Design review of the part built by this model. Coordinates are the model's own, in mm. A direction names the side the tool comes from. Round coordinates to 2 decimals unless told otherwise and drop trailing zeros. Order: outer loops, then holes, each group sorted by start corner. A loop starts at its lowest first (then second) coordinate and runs counter-clockwise, first axis right, second up.
from build123d import *

# Parameters (mm, degrees)
SKETCH1_W           = 32
SKETCH1_H           = 45
BOSS_EXTRUDE1_DEPTH = 8
CUT_EXTRUDE1_DEPTH  = 29.744564704
CUT_EXTRUDE2_DEPTH  = 3.3
FILLET1_R           = 3


with BuildPart() as part:
    # Sketch1 → Boss-Extrude1 (new body)
    with BuildSketch(Plane.XY):
        Rectangle(SKETCH1_W, SKETCH1_H)
    extrude(amount=BOSS_EXTRUDE1_DEPTH)

    # Sketch5 → Cut-Extrude1 (cut, through all)
    with BuildSketch(Plane.XY.offset(8)):
        with BuildLine():
            Line((-8, 1.75), (8, 1.75))
            ThreePointArc((8, 1.75), (9.75, 0), (8, -1.75))
            Line((8, -1.75), (-8, -1.75))
            ThreePointArc((-8, -1.75), (-9.75, 0), (-8, 1.75))
        make_face()
    extrude(amount=-CUT_EXTRUDE1_DEPTH, mode=Mode.SUBTRACT)

    # Sketch6 → Cut-Extrude2 (cut)
    with BuildSketch(Plane.XY.offset(8)):
        with BuildLine():
            Line((-8, 3), (8, 3))
            ThreePointArc((8, 3), (11, 0), (8, -3))
            Line((8, -3), (-8, -3))
            ThreePointArc((-8, -3), (-11, 0), (-8, 3))
        make_face()
    extrude(amount=-CUT_EXTRUDE2_DEPTH, mode=Mode.SUBTRACT)

    # Fillet1
    fillet1_edges = [part.edges().sort_by_distance(p)[0] for p in [
        (-16, 22.5, 4),
        (16, 22.5, 4),
        (16, -22.5, 4),
        (-16, -22.5, 4),
    ]]
    fillet(fillet1_edges, radius=FILLET1_R)


solid = part.part
1) To check wall thickness, follow line 1 along Y through (x, z) = (-3, 6.5); line 2 along Y through (x, z) = (5, 2.5); line 3 along X through (y, z) = (0, 6.5). State the ranges of each line that lie inside material, in increasing order.
Results:
line 1: y = -22.5 to -3, 3 to 22.5
line 2: y = -22.5 to -1.75, 1.75 to 22.5
line 3: x = -16 to -11, 11 to 16
2) Take a section at C-C on x = -5. Give the boundary of the cut face in (y, z).
Results:
outline: (-22.5, 0) - (-1.75, 0) - (-1.75, 4.7) - (-3, 4.7) - (-3, 8) - (-22.5, 8) - close; (1.75, 0) - (22.5, 0) - (22.5, 8) - (3, 8) - (3, 4.7) - (1.75, 4.7) - close
3) Clearance check with a flat-ended pin moving along its axis: P1, Ø3, axis at x = 2.5, y = -0.5, coming from the +Z side. State where the tip first meets the part, or that it passes through.
Results:
P1: stops at z = 4.7
4) Take a section at A-A on z = 7.5. Give the boundary of the cut face in (x, y).
Results:
outline: (-16, -19.5) arc R3 ccw to (-13, -22.5) - (13, -22.5) arc R3 ccw to (16, -19.5) - (16, 19.5) arc R3 ccw to (13, 22.5) - (-13, 22.5) arc R3 ccw to (-16, 19.5) - close; hole (-8, -3) - (8, -3) arc R3 ccw to (8, 3) - (-8, 3) arc R3 ccw to start
5) Take a section at D-D on z = 2.75. Give the boundary of the cut face in (x, y).
Results:
outline: (-16, -19.5) arc R3 ccw to (-13, -22.5) - (13, -22.5) arc R3 ccw to (16, -19.5) - (16, 19.5) arc R3 ccw to (13, 22.5) - (-13, 22.5) arc R3 ccw to (-16, 19.5) - close; hole (-8, -1.75) - (8, -1.75) arc R1.75 ccw to (8, 1.75) - (-8, 1.75) arc R1.75 ccw to start
6) The part is to be moulded in two halves that separate along Y. For faces 4 (the face through (16, 0, 4)), 5 (the face through (15.1, 21.64, 4.06)), 6 (the face through (0, -22.5, 4)), 7 (the face through (0, 3, 6)), say which applies: released by +Y, released by -Y, zero draft, split by the parting line, or undercut.
Results:
face 4: zero draft
face 5: released by +Y
face 6: released by -Y
face 7: undercut
7) Take a section at B-B on y = 0. Give the boundary of the cut face in (x, z), plus the area to 4 significant figures.
Results:
outline: (-16, 0) - (-9.75, 0) - (-9.75, 4.7) - (-11, 4.7) - (-11, 8) - (-16, 8) - close; (9.75, 0) - (16, 0) - (16, 8) - (11, 8) - (11, 4.7) - (9.75, 4.7) - close
area: 91.75 mm2
8) For faces 1 (the face through (-11, 0, 6)), 2 (the face through (-9.75, -0.04, 2.38)), 3 (the face through (-16, 0, 4)), list the 3-axis set-ups (+Z, -Z, +X, -X, +Y, -Y) from which the entire face can be reached by the end or side of a thin tool; tool diameter is ignored.
Results:
face 1: +Z
face 2: +Z, -Z
face 3: +Z, -Z, -X, +Y, -Y
